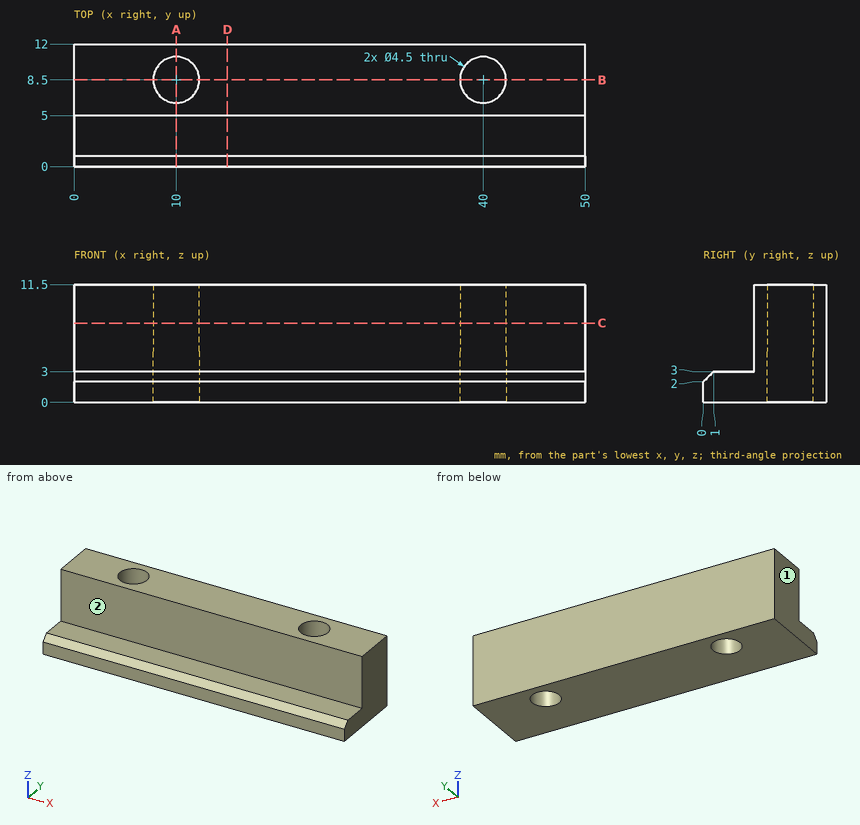
Could you check a few things on this drawing? It's one solid part, dimensions in mm from its lowest x, y, z. A direction names the side the tool comes from. Give positions to 0.01 mm unless a question says otherwise; leave off trailing zeros. Order: outer loops, then holes, each group sorted by start corner. A loop starts at its lowest first (then second) coordinate and runs counter-clockwise, first axis right, second up.
1. For pin 1 (4 mm diameter, centred on x = 13.5, z = 6, fed in from -Y); pin 2 (4.5 mm diameter, centred on x = 21, y = 2.5, fed in from +Z), each with a flat end and sliding along its axis, tell me the tip position at first contact or that it passes through.
Answers below:
pin 1: stops at y = 5
pin 2: stops at z = 3
2. Suppose I cut it at C-C (z = 7.75). Write out the boundary of the cut face in (x, y).
Answers below:
outline: (0, 5) - (50, 5) - (50, 12) - (0, 12) - close; hole circle Ø4.5 at (10, 8.5); hole circle Ø4.5 at (40, 8.5)
3. Suppose I cut it at B-B (y = 8.5). Write out the boundary of the cut face in (x, z), plus the area to 4 significant figures.
Answers below:
outline: (0, 0) - (7.75, 0) - (7.75, 11.5) - (0, 11.5) - close; (12.25, 0) - (37.75, 0) - (37.75, 11.5) - (12.25, 11.5) - close; (42.25, 0) - (50, 0) - (50, 11.5) - (42.25, 11.5) - close
area: 471.5 mm2
4. Suppose I cut it at A-A (x = 10). Write out the boundary of the cut face in (y, z).
Answers below:
outline: (0, 0) - (6.25, 0) - (6.25, 11.5) - (5, 11.5) - (5, 3) - (1, 3) - (0, 2) - close; (10.75, 0) - (12, 0) - (12, 11.5) - (10.75, 11.5) - close
5. Which directions (+Z, -Z, +X, -X, +Y, -Y) give clear straight access to the entire face, cutting with the end or side of a thin tool? Please do the marked faces 1 and 2.
Answers below:
face 1: +Z, -Z, -X, +Y, -Y
face 2: +Z, +X, -X, -Y
6. I need wall thicknesses on L1, parallel to Y at x = 10, z = 6.75; L2, parallel to Y at x = 40, z = 1.45; L3, parallel to Y at x = 24, z = 10.5. Which ranges of each line are inside material? Lowest first, please.
Answers below:
L1: y = 5 to 6.25, 10.75 to 12
L2: y = 0 to 6.25, 10.75 to 12
L3: y = 5 to 12
7. Suppose I cut it at D-D (x = 15). Write out the boundary of the cut face in (y, z).
Answers below:
outline: (0, 0) - (12, 0) - (12, 11.5) - (5, 11.5) - (5, 3) - (1, 3) - (0, 2) - close
